from build123d import *

# Parameters (mm, degrees)
SKETCH_1_W          = 330
SKETCH_1_H          = 200
EXTRUDE_1_DEPTH     = 1.5
SKETCH_2_R          = 3.2
CUT_EXTRUDE_1_DEPTH = 11.5


with BuildPart() as part:
    # 草图1 → 凸台-拉伸1 (new, symmetric)
    with BuildSketch(Plane.XY):
        Rectangle(SKETCH_1_W, SKETCH_1_H)
    extrude(amount=EXTRUDE_1_DEPTH, both=True)

    # 草图2 → 切除-拉伸1 (cut, symmetric)
    with BuildSketch(Plane.XY):
        with Locations((-145, -80)):
            Circle(SKETCH_2_R)
        with Locations((145, 80)):
            Circle(SKETCH_2_R)
    extrude(amount=CUT_EXTRUDE_1_DEPTH, both=True, mode=Mode.SUBTRACT)


solid = part.part
Here's how the part is built. I have some questions about the finished solid (model axes, mm). Coordinates: 2 decimals unless noted, no trailing zeros. Loops run counter-clockwise (first coordinate to the right, second up) from the corner with the lowest first, then second, coordinate; pieces in that order, holes last. Notation, with made-up numbers: (55, 34) -> (104, 34) arc R8 cw to (104, 43) -> close; hole circle Ø1 at (48, 81). An arc over 180 degrees is marked (long way). Use one line per item in the form item = value. Start each with the question number.
(1) We'd pull the mould along X, two halves only. Please class faces 1 (the face through (147.956, 78.774, 0.021)), 2 (the face through (-2, 1, 1.5)): pulls with the +X half, pulls with the -X half, needs draft (parallel to the pull), parting line crosses it, or undercut.
(2) Will this pin go through, and if not, where does the flat tip stop? pin 1 (4 mm diameter, centred on x = -145, y = -80, fed in from -Z).
(3) Please list where these lines run through material, in increasing order: line 1 along Y through (x, z) = (-145, 0.6); line 2 along Y through (x, z) = (145, 0.7); line 3 along X through (y, z) = (-80, -0.4).
(4) If we section it at B-B (y = 80): Please give me the cut outline in (x, z), then the cut area to 3 significant figures.
(5) If we section it at A-A (x = -145): Please give me the cut outline in (y, z), then the cut area to 3 significant figures.
Verdict:
q1.face_1 = undercut
q1.face_2 = needs draft
q2.pin_1 = through
q3.line_1 = -100 to -83.2, -76.8 to 100
q3.line_2 = -100 to 76.8, 83.2 to 100
q3.line_3 = -165 to -148.2, -141.8 to 165
q4.outline = (-165, -1.5) -> (141.8, -1.5) -> (141.8, 1.5) -> (-165, 1.5) -> close; (148.2, -1.5) -> (165, -1.5) -> (165, 1.5) -> (148.2, 1.5) -> close
q4.area = 971 mm²
q5.outline = (-100, -1.5) -> (-83.2, -1.5) -> (-83.2, 1.5) -> (-100, 1.5) -> close; (-76.8, -1.5) -> (100, -1.5) -> (100, 1.5) -> (-76.8, 1.5) -> close
q5.area = 581 mm²
